CAD build for the part. Positions are in the model's coordinates, mm. A direction names the side the tool comes from. Round coordinates to 2 decimals unless told otherwise and drop trailing zeros. Loops run counter-clockwise (first coordinate to the right, second up) from the corner with the lowest first, then second, coordinate; pieces in that order, holes last.
```python
from build123d import *

# Parameters (mm, degrees)
SKETCH1_R               = 205
SKETCH1_R_2             = 125
BOSS_EXTRUDE1_DEPTH     = 2300
BOSS_EXTRUDE2_START     = 400
SKETCH2_R               = 205
BOSS_EXTRUDE2_DEPTH     = 400
CUT_EXTRUDE1_DEPTH      = 5000
CUT_EXTRUDE1_DEPTH_BACK = 4000
SKETCH3_R               = 100
CHAMFER1_SIZE           = 30


with BuildPart() as part:
    # Sketch1 → Boss-Extrude1 (new body)
    with BuildSketch(Plane(origin=(0, 0, 0), x_dir=(1, 0, 0), z_dir=(0, 1, 0))):
        with Locations(Location((0, 0, 0), (0, 0, 270))):
            Circle(SKETCH1_R)
        with Locations(Location((0, 0, 0), (0, 0, 270))):
            Circle(SKETCH1_R_2, mode=Mode.SUBTRACT)
    extrude(amount=BOSS_EXTRUDE1_DEPTH)

    # Sketch2 → Boss-Extrude2 (add)
    with BuildSketch(Plane.XZ.offset(BOSS_EXTRUDE2_START)):
        with Locations(Location((0, 0, 0), (0, 0, 270))):
            Circle(SKETCH2_R)
    extrude(amount=-BOSS_EXTRUDE2_DEPTH)

    # Sketch3 → Cut-Extrude1 (cut, two sides: drawn at the far end of the back side and taken through both)
    with BuildSketch(Plane(origin=(0, 0, 0), x_dir=(0, 0, -1), z_dir=(1, 0, 0)).offset(-CUT_EXTRUDE1_DEPTH_BACK)):
        with Locations(Location((0, -260.843725605, 0), (0, 0, 180))):
            Circle(SKETCH3_R)
    extrude(amount=CUT_EXTRUDE1_DEPTH + CUT_EXTRUDE1_DEPTH_BACK, mode=Mode.SUBTRACT)

    # Chamfer1
    chamfer1_edges = [part.edges().sort_by_distance(p)[0] for p in [
        (0, 2300, -205),
    ]]
    chamfer(chamfer1_edges, length=CHAMFER1_SIZE)


solid = part.part
```
Item 1: Flat gauge pins, fed straight in: P1, Ø6, axis at y = 1672.5, z = -10, coming from the +X side; P2, Ø1.5, axis at y = 17, z = 68.5, coming from the +X side; P3, Ø3, axis at y = 1551.5, z = 15, coming from the -X side (3 decimals). Where does each tip first touch, or does it go through?
Answers follow:
P1: stops at x = 204.88
P2: stops at x = 193.48
P3: stops at x = -204.555
Item 2: Cut at A-A, the plane z = 0. Give the cut face in (x, y), plus the area to 3 significant figures.
Answers follow:
outline: (-205, -400) - (205, -400) - (205, -360.84) - (-205, -360.84) - close; (-205, -160.84) - (205, -160.84) - (205, 2270) - (175, 2300) - (125, 2300) - (125, 0) - (-125, 0) - (-125, 2300) - (-175, 2300) - (-205, 2270) - close
area: 449,000 mm2
Item 3: Cut at C-C, the plane x = 0. Give the cut face in (y, z), plus the area to 3 significant figures.
Answers follow:
outline: (-400, -205) - (2270, -205) - (2300, -175) - (2300, -125) - (0, -125) - (0, 125) - (2300, 125) - (2300, 175) - (2270, 205) - (-400, 205) - close; hole circle Ø200 at (-260.84, 0)
area: 500,000 mm2
Item 4: 3-axis set-ups, long thin cutter, end or side, ignore diameter. For faces 1 (the cylindrical face through (5.5, 1133.9, -124.88)), 2 (the cylindrical face through (-2.87, -290.881, 95.382)): which of +Z, -Z, +X, -X, +Y, -Y reach the whole face in a straight line?
Answers follow:
face 1: +Y
face 2: +X, -X
Item 5: Two-plate mould, pull along X, no slides. Class faces 3 (the flat face through (2, 0, 2)), 4 (the flat face through (3, -400, 3)), 5 (the conical face through (-107.371, 2298.543, -140.03)): released by +X, released by -X, zero draft, split by the parting line, or undercut.
Answers follow:
face 3: undercut
face 4: zero draft
face 5: split by the parting line
Item 6: Cut at B-B, the plane y = 1522.5. Give the cut face in (x, z).
Answers follow:
outline: circle Ø410 at (0, 0); hole circle Ø250 at (0, 0)
Item 7: Probe line 1 (X direction, y = 363, z = -7); line 2 (X direction, y = 159.5, z = -1.5); line 3 (Y direction, x = -53, z = 0). List the from-to ranges inside material, lowest first.
Answers follow:
line 1: x = -204.88 to -124.8, 124.8 to 204.88
line 2: x = -204.99 to -124.99, 124.99 to 204.99
line 3: y = -400 to -360.84, -160.84 to 0
